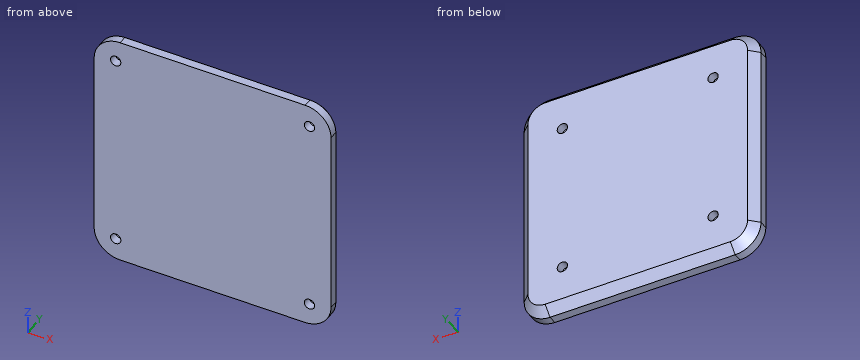
```python
from build123d import *

# Parameters (mm, degrees)
BASE_PLATE_PROFILE_275X275_W       = 275
BASE_PLATE_PROFILE_275X275_H       = 275
BASE_PLATE_275X275X20_DEPTH        = 20
CORNER_FILLETS_R30_R               = 30
EDGE_CHAMFER_10X45_SIZE            = 10
DOWEL_HOLES_12_ON_175_SQUARE_D     = 12
DOWEL_HOLES_12_ON_175_SQUARE_DEPTH = 10
DOWEL_HOLES_12_ON_175_SQUARE_TIP   = 3.605163714
DOWEL_HOLES_12_ON_225_SQUARE_D     = 12
DOWEL_HOLES_12_ON_225_SQUARE_DEPTH = 10
DOWEL_HOLES_12_ON_225_SQUARE_TIP   = 3.605163714


with BuildPart() as part:
    # Base Plate Profile 275x275 → Base Plate 275x275x20 (new body)
    with BuildSketch(Plane(origin=(0, 0, 0), x_dir=(1, 0, 0), z_dir=(0, 1, 0))):
        Rectangle(BASE_PLATE_PROFILE_275X275_W, BASE_PLATE_PROFILE_275X275_H)
    extrude(amount=BASE_PLATE_275X275X20_DEPTH)

    # Corner Fillets R30
    corner_fillets_r30_edges = [part.edges().sort_by_distance(p)[0] for p in [
        (-137.5, 10, 137.5),
        (-137.5, 10, -137.5),
        (137.5, 10, -137.5),
        (137.5, 10, 137.5),
    ]]
    fillet(corner_fillets_r30_edges, radius=CORNER_FILLETS_R30_R)

    # Edge Chamfer 10x45
    edge_chamfer_10x45_edges = [part.edges().sort_by_distance(p)[0] for p in [
        (0, 20, -137.5),
        (137.5, 20, 0),
        (0, 20, 137.5),
        (-137.5, 20, 0),
        (-128.713203436, 20, 128.713203436),
        (128.713203436, 20, 128.713203436),
        (-128.713203436, 20, -128.713203436),
        (128.713203436, 20, -128.713203436),
    ]]
    chamfer(edge_chamfer_10x45_edges, length=EDGE_CHAMFER_10X45_SIZE)

    # Dowel Holes Ø12 on 175 Square
    with Locations(Plane(origin=(-87.5, 20, -87.5), x_dir=(0, 0, 1), z_dir=(0, 1, 0))):
        with Locations((0, 0), (0, 175), (175, 175), (175, 0)):
            Hole(DOWEL_HOLES_12_ON_175_SQUARE_D / 2, depth=DOWEL_HOLES_12_ON_175_SQUARE_DEPTH)
            with Locations((0, 0, -(DOWEL_HOLES_12_ON_175_SQUARE_DEPTH + DOWEL_HOLES_12_ON_175_SQUARE_TIP / 2))):  # 118° drill point
                Cone(0, DOWEL_HOLES_12_ON_175_SQUARE_D / 2, DOWEL_HOLES_12_ON_175_SQUARE_TIP, mode=Mode.SUBTRACT)

    # Dowel Holes Ø12 on 225 Square
    with Locations(Plane(origin=(-112.5, 0, 112.5), x_dir=(0, 0, -1), z_dir=(0, -1, 0))):
        with Locations((0, 0), (0, 225), (225, 225), (225, 0)):
            Hole(DOWEL_HOLES_12_ON_225_SQUARE_D / 2, depth=DOWEL_HOLES_12_ON_225_SQUARE_DEPTH)
            with Locations((0, 0, -(DOWEL_HOLES_12_ON_225_SQUARE_DEPTH + DOWEL_HOLES_12_ON_225_SQUARE_TIP / 2))):  # 118° drill point
                Cone(0, DOWEL_HOLES_12_ON_225_SQUARE_D / 2, DOWEL_HOLES_12_ON_225_SQUARE_TIP, mode=Mode.SUBTRACT)


solid = part.part
```
Can you work these out from the model? Positions are in its coordinate system, mm. Round coordinates to 2 decimals unless told otherwise and drop trailing zeros. Loops run counter-clockwise (first coordinate to the right, second up) from the corner with the lowest first, then second, coordinate; pieces in that order, holes last. Notation, with made-up numbers: M 3.5,-28.75 L 14.5,-28.75 A23 cw 14.5,9.25 Z; hole C -26,23.25 d11. An arc over 180 degrees is marked long. Write item = value, one per line. Start each with the question number.
(1) I'm going to push flat-ended pins straight in: P1, Ø8, axis at x = -58.5, y = 15, coming from the +Z side; P2, Ø10, axis at x = -12.5, y = 15.5, coming from the -Z side; P3, Ø11, axis at x = -87.5, z = -87.5, coming from the +Y side. Where does each tip first touch, or does it pass through?
(2) I need wall thicknesses on line 1 along X through (y, z) = (15, -87.5); line 2 along X through (y, z) = (18, -87.5); line 3 along Z through (x, y) = (112.5, 6.25). Which ranges of each line are inside material? Lowest first, please.
(3) Suppose I cut it at B-B on x = 18. Write out the boundary of the cut face in (y, z).
(4) Suppose I cut it at A-A on z = 97. Write out the boundary of the cut face in (x, y), plus the area to 3 significant figures.
Answer block:
q1.P1 = 136.5
q1.P2 = -137
q1.P3 = 9.7
q2.line_1 = -132.5 to -93.5, -81.5 to 81.5, 93.5 to 132.5
q2.line_2 = -129.5 to -93.5, -81.5 to 81.5, 93.5 to 129.5
q2.line_3 = -137.08 to -118.5, -106.5 to 106.5, 118.5 to 137.08
q3.outline = M 0,-137.5 L 10,-137.5 L 20,-127.5 L 20,127.5 L 10,137.5 L 0,137.5 Z
q4.outline = M -137.5,0 L 137.5,0 L 137.5,10 L 127.5,20 L -127.5,20 L -137.5,10 Z
q4.area = 5,400 mm²
